```python
from build123d import *

# Parameters (mm, degrees)
EXTRUDE_1_DEPTH     = 20
SKETCH_4_R          = 7
CUT_EXTRUDE_1_DEPTH = 20
SKETCH_5_R          = 4.5
CUT_EXTRUDE_2_DEPTH = 20
CHAMFER_1_SIZE      = 2
CHAMFER_2_SIZE      = 0.5


with BuildPart() as part:
    # 草图2 → 凸台-拉伸1 (new body)
    with BuildSketch(Plane.XY):
        with BuildLine():
            Line((0, 0), (0, 25))
            Line((0, 25), (70, 25))
            ThreePointArc((70, 25), (88.959441577, 24.682639084), (104.868973518, 35))
            Line((104.868973518, 35), (115, 35))
            Line((115, 35), (115, 0))
            Line((115, 0), (0, 0))
        make_face()
    extrude(amount=EXTRUDE_1_DEPTH)

    # 草图4 → 切除-拉伸1 (cut)
    with BuildSketch(Plane(origin=(0, 35, 0), x_dir=(1, 0, 0), z_dir=(0, 1, 0))):
        with Locations(Location((42.5, -10, 0), (0, 0, 180))):
            Circle(SKETCH_4_R)
        with Locations(Location((72.5, -10, 0), (0, 0, 180))):
            Circle(SKETCH_4_R)
    extrude(amount=-CUT_EXTRUDE_1_DEPTH, mode=Mode.SUBTRACT)

    # 草图5 → 切除-拉伸2 (cut)
    with BuildSketch(Plane(origin=(0, 15, 0), x_dir=(1, 0, 0), z_dir=(0, 1, 0))):
        with Locations(Location((42.5, -10, 0), (0, 0, 180))):
            Circle(SKETCH_5_R)
        with Locations(Location((72.5, -10, 0), (0, 0, 180))):
            Circle(SKETCH_5_R)
    extrude(amount=-CUT_EXTRUDE_2_DEPTH, mode=Mode.SUBTRACT)

    # 倒角1
    chamfer_1_edges = [part.edges().sort_by_distance(p)[0] for p in [
        (0, 12.5, 20),
        (0, 12.5, 0),
        (115, 17.5, 20),
        (115, 17.5, 0),
    ]]
    chamfer(chamfer_1_edges, length=CHAMFER_1_SIZE)

    # 倒角2
    chamfer_2_edges = [part.edges().sort_by_distance(p)[0] for p in [
        (88.959441577, 24.682639084, 20),
        (36, 25, 20),
        (108.934486759, 35, 20),
        (108.934486759, 35, 0),
        (36, 25, 0),
        (88.959441577, 24.682639084, 0),
    ]]
    chamfer(chamfer_2_edges, length=CHAMFER_2_SIZE)


solid = part.part
```
Check sheet for the modelled part. Datum: model origin and axes. Units: mm. A direction names the side the tool comes from. Coordinates: 2 decimals unless noted, no trailing zeros. Loops run counter-clockwise (first coordinate to the right, second up) from the corner with the lowest first, then second, coordinate; pieces in that order, holes last.
1) Gauge pin test, flat ends, axial feed: pin 1 (9.5 mm diameter, centred on x = 32.5, z = 5.5, fed in from +Y); pin 2 (4 mm diameter, centred on x = 39, z = 11, fed in from +Y). Record the tip position at first contact, or that the pin passes through.
2) Release check for a two-part mould opening along X. For faces 1 (the face through (66.034, 20.07, 7.319)), 2 (the face through (114, 18, 1)), 3 (the face through (36.034, 20.07, 7.319)), 4 (the face through (58, 14, 20)) record: released by +X, released by -X, zero draft, split by the parting line, or undercut.
3) Sectioned sample at B-B (x = 41.5). Record the boundary of the cut face in (y, z), and give its area (3 significant figures).
4) Sectioned sample at C-C (z = 10). Record the boundary of the cut face in (x, y).
5) Access from +Z, -Z, +X, -X, +Y, -Y to the whole of each face (thin tool, end or side, straight path). Record for faces 5 (the face through (73, 15, 5)), 6 (the face through (38.208, 7.605, 11.352)), 7 (the face through (35, 25, 10)).
6) Material ranges on probe 1 along Z at (x, y) = (72, 17); probe 2 along Z at (x, y) = (72.5, 9.5); probe 3 along X at (y, z) = (17, 6.5), recorded low to high.
7) Sectioned sample at A-A (y = 12). Record the boundary of the cut face in (x, z), and give its area (3 significant figures).
8) Sectioned sample at D-D (x = 22). Record the boundary of the cut face in (y, z).
Check sheet entries:
1. pin 1: stops at y = 25
1. pin 2: stops at y = 15
2. face 1: undercut
2. face 2: released by +X
2. face 3: undercut
2. face 4: zero draft
3. outline: (0, 0) - (24.5, 0) - (25, 0.5) - (25, 3.07) - (15, 3.07) - (15, 5.61) - (0, 5.61) - close; (0, 14.39) - (15, 14.39) - (15, 16.93) - (25, 16.93) - (25, 19.5) - (24.5, 20) - (0, 20) - close
3. area: 230 mm2
4. outline: (0, 0) - (38, 0) - (38, 15) - (35.5, 15) - (35.5, 25) - (0, 25) - close; (47, 0) - (68, 0) - (68, 15) - (65.5, 15) - (65.5, 25) - (49.5, 25) - (49.5, 15) - (47, 15) - close; (77, 0) - (115, 0) - (115, 35) - (104.87, 35) arc R32.5 cw to (79.5, 23.43) - (79.5, 15) - (77, 15) - close
5. face 5: +Y
5. face 6: +Y, -Y
5. face 7: +Z, -Z, -X, +Y
6. probe 1: z = 0 to 3.02, 16.98 to 20
6. probe 2: z = 0 to 5.5, 14.5 to 20
6. probe 3: x = 0 to 36.44, 48.56 to 66.44, 78.56 to 115
7. outline: (0, 2) - (2, 0) - (113, 0) - (115, 2) - (115, 18) - (113, 20) - (2, 20) - (0, 18) - close; hole circle Ø9 at (42.5, 10); hole circle Ø9 at (72.5, 10)
7. area: 2,160 mm2
8. outline: (0, 0) - (24.5, 0) - (25, 0.5) - (25, 19.5) - (24.5, 20) - (0, 20) - close
